Verification items for this drawing (mm, ordinates from the low corner). A direction names the side the tool comes from. Coordinates: 2 decimals unless noted, no trailing zeros. Loops run counter-clockwise (first coordinate to the right, second up) from the corner with the lowest first, then second, coordinate; pieces in that order, holes last. Notation, with made-up numbers: M 15.25,41 L 53.25,41 A22 cw 53.25,71 Z; hole C 68.25,88.5 d4. An arc over 180 degrees is marked long. Return JSON: item names as keys, results as strings.
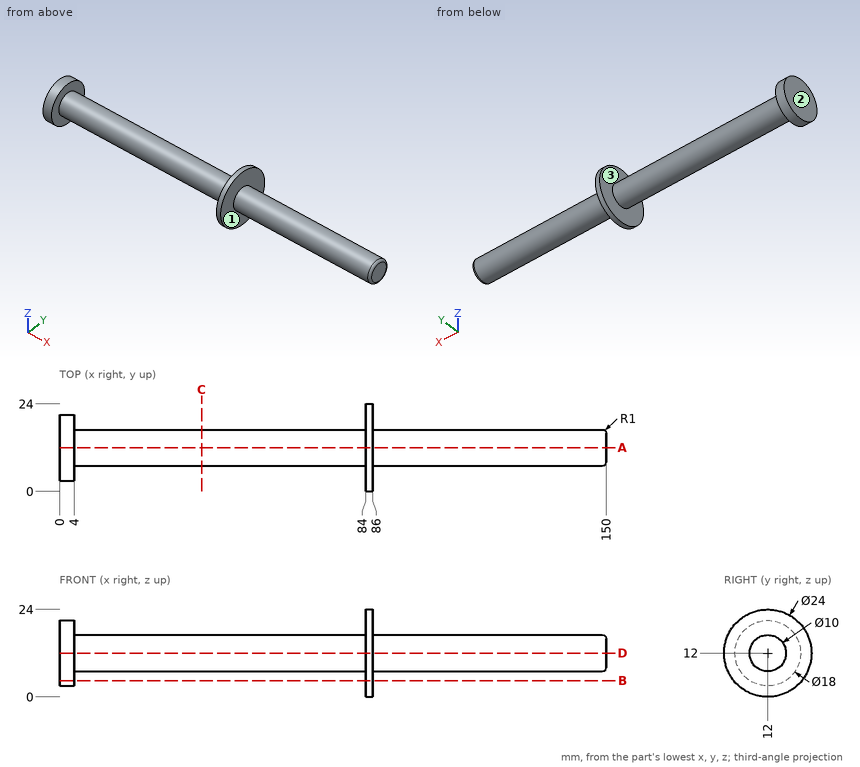
1) Section check C-C on x = 39. Record the cut outline in (y, z), then the cut area to 3 significant figures.
Answers:
{"outline": "C 12,12 d10", "area": "78.5 mm²"}
2) Set-up check for the marked faces 1, 2 and 3: record each of +Z, -Z, +X, -X, +Y, -Y from which the full face is reachable in a straight line by a thin tool's end or side.
Answers:
{"face 1": "+X", "face 2": "+Z, -Z, -X, +Y, -Y", "face 3": "none"}
3) Section check B-B on z = 4.5. Record the cut outline in (x, y), then the cut area to 3 significant figures.
Answers:
{"outline": "M 0,7.03 L 4,7.03 L 4,16.97 L 0,16.97 Z; M 84,2.63 L 86,2.63 L 86,21.37 L 84,21.37 Z", "area": "77.3 mm²"}
4) Scan lines: line 1 along X through (y, z) = (5.25, 7); line 2 along X through (y, z) = (19.25, 5.25); line 3 along Z through (x, y) = (9, 7.75). Record each from-to range of solid material in increasing order. Write a range as [from, to].
Answers:
{"line 1": "[0, 4], [84, 86]", "line 2": "[84, 86]", "line 3": "[9.37, 14.63]"}
5) Go/stop test with flat-tipped pins: pin 1 Ø4 at (x, y) = (107, 7) entering from -Z; pin 2 Ø8 at (x, z) = (109.5, 9.5) entering from -Y; pin 3 Ø2 at (y, z) = (20.5, 17.5) entering from +X. Record where each tip stops, or that it passes through.
Answers:
{"pin 1": "z = 8", "pin 2": "y = 7", "pin 3": "x = 86"}
6) Section check A-A on y = 12. Record the cut outline in (x, z), then the cut area to 3 significant figures.
Answers:
{"outline": "M 0,3 L 4,3 L 4,7 L 84,7 L 84,0 L 86,0 L 86,7 L 149,7 A1 ccw 150,8 L 150,16 A1 ccw 149,17 L 86,17 L 86,24 L 84,24 L 84,17 L 4,17 L 4,21 L 0,21 Z", "area": "1,560 mm²"}
